```python
from build123d import *

# Parameters (mm, degrees)
BASE_BLOCK_DEPTH      = 20
BASE_RECESS_CUT_DEPTH = 75
HUB_CIRCLE_SKETCH_R   = 20
BEARING_HUB_DEPTH     = 44
SUPPORT_WEB_DEPTH     = 24
SIDE_WINDOW_CUT_DEPTH = 24
BEARING_BORE_SKETCH_R = 8
BEARING_BORE_DEPTH    = 57
SIDE_RIB_DEPTH        = 20


with BuildPart() as part:
    # Base Profile Sketch → Base Block (new body)
    with BuildSketch(Plane(origin=(0, 0, 0), x_dir=(1, 0, 0), z_dir=(0, 1, 0))):
        Polygon((30, 0), (30, 45), (-30, 45), (-30, -45), (30, -45), align=None)
    extrude(amount=BASE_BLOCK_DEPTH)

    # Base Recess Sketch → Base Recess Cut (cut)
    with BuildSketch(Plane(origin=(30, 0, 0), x_dir=(0, 0, -1), z_dir=(1, 0, 0))):
        Polygon((38, 20), (45, 0), (45, 20), align=None)
        Polygon((-38, 20), (-45, 0), (-45, 20), align=None)
    extrude(amount=-BASE_RECESS_CUT_DEPTH, mode=Mode.SUBTRACT)



with BuildPart() as body_2:
    # Hub Circle Sketch → Bearing Hub (new body)
    with BuildSketch(Plane(origin=(12, 0, 0), x_dir=(0, 0, -1), z_dir=(1, 0, 0))):
        with Locations((0, 50)):
            Circle(HUB_CIRCLE_SKETCH_R)
    extrude(amount=-BEARING_HUB_DEPTH)


with BuildPart() as part_1:
    add(part.part)

    add(body_2.part)  # Support Web merges body 2
    # Support Web Sketch → Support Web (add)
    with BuildSketch(Plane(origin=(2, 0, 0), x_dir=(0, 0, -1), z_dir=(1, 0, 0))):
        with BuildLine():
            Line((25, 20), (-25, 20))
            Line((-25, 20), (-38, 20))
            Line((-38, 20), (-25, 58))
            Line((-25, 58), (-18.33030278, 58))
            ThreePointArc((-18.33030278, 58), (0, 30), (18.33030278, 58))
            Line((18.33030278, 58), (25, 58))
            Line((25, 58), (38, 20))
            Line((38, 20), (25, 20))
        make_face()
    extrude(amount=-SUPPORT_WEB_DEPTH)

    # Side Window Sketch → Side Window Cut (cut)
    with BuildSketch(Plane(origin=(2, 0, 0), x_dir=(0, 0, -1), z_dir=(1, 0, 0))):
        with BuildLine():
            Line((-8, 68.33030278), (-8, 58))
            Line((-8, 58), (-18.33030278, 58))
            ThreePointArc((-18.33030278, 58), (-14.142135624, 64.142135624), (-8, 68.33030278))
        make_face()
    side_window_cut = extrude(amount=-SIDE_WINDOW_CUT_DEPTH, mode=Mode.SUBTRACT)

    # Side Window Mirror: Side Window Cut across plane
    add(side_window_cut.mirror(Plane.XY), mode=Mode.SUBTRACT)

    # Bearing Bore Sketch → Bearing Bore (cut)
    with BuildSketch(Plane(origin=(12, 0, 0), x_dir=(0, 0, -1), z_dir=(1, 0, 0))):
        with Locations((0, 50)):
            Circle(BEARING_BORE_SKETCH_R)
    extrude(amount=-BEARING_BORE_DEPTH, mode=Mode.SUBTRACT)

    # Side Rib Sketch → Side Rib (add)
    with BuildSketch(Plane.XY.offset(45)):
        Polygon((-10, 7), (-2, 7), (-2, 45), (-18, 45), (-18, 7), align=None)
    side_rib = extrude(amount=-SIDE_RIB_DEPTH)

    # Side Rib Mirror: Side Rib across plane
    add(side_rib.mirror(Plane.XY))


solid = part_1.part
```
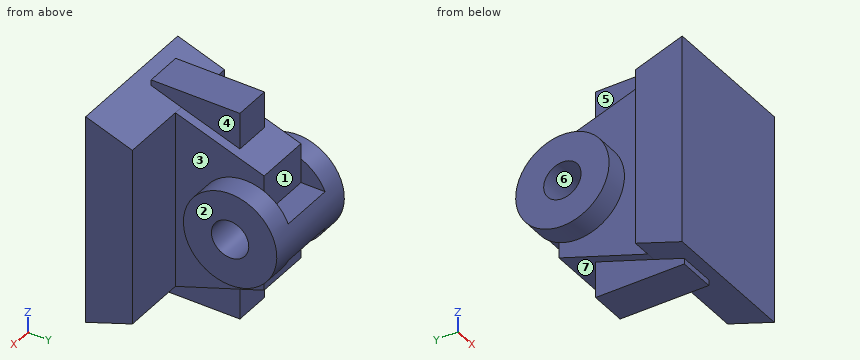
Design review of the part built by this model. Coordinates are the model's own, in mm. Face numbers are marked on the shaded views. A direction names the side the tool comes from. Give positions to 0.01 mm unless a question says otherwise; leave off trailing zeros. Write each loop counter-clockwise with the first axis right and the second up, starting at its lowest first coordinate (ties: lowest second). Pieces come first, ordered by that corner, then holes.
(1) Add section A-A (y = 16). Give the boundary of the cut face in (x, z).
Checked values:
outline: (-30, -39.4) - (-18, -39.4) - (-18, -45) - (-2, -45) - (-2, -39.4) - (30, -39.4) - (30, 39.4) - (-2, 39.4) - (-2, 45) - (-18, 45) - (-18, 39.4) - (-30, 39.4) - close
(2) Mouldability with a two-part tool opening along Y and no side actions: class the marked faces 5, 6 and 7 as +Y half, -Y half, draft (parallel to the pull), parting line (faces both ways), or undercut.
Checked values:
face 5: draft
face 6: undercut
face 7: +Y half
(3) Clearance check with flat-ended pins moving along their axes: pin 1 Ø10 at (x, z) = (9.5, 10) entering from +Y; pin 2 Ø6 at (y, z) = (38, -31.5) entering from +X; pin 3 Ø17 at (x, z) = (-9, -38.5) entering from +Y. State where each tip first meets the part, or that it passes through.
Checked values:
pin 1: stops at y = 69.36
pin 2: stops at x = 2
pin 3: stops at y = 45
(4) Add section C-C (y = 50). Give the boundary of the cut face in (x, z).
Checked values:
outline: (-32, -20) - (-22, -20) - (-22, -27.74) - (2, -27.74) - (2, -20) - (12, -20) - (12, -8) - (-32, -8) - close; (-32, 8) - (12, 8) - (12, 20) - (2, 20) - (2, 27.74) - (-22, 27.74) - (-22, 20) - (-32, 20) - close
(5) Add section B-B (z = 0). Give the boundary of the cut face in (x, y), and give its area (3 significant figures).
Checked values:
outline: (-32, 30) - (-22, 30) - (-22, 20) - (-30, 20) - (-30, 0) - (30, 0) - (30, 20) - (2, 20) - (2, 30) - (12, 30) - (12, 42) - (-32, 42) - close; (-32, 58) - (12, 58) - (12, 70) - (-32, 70) - close
area: 2,500 mm2
(6) Tool access review of the marked faces 1, 2, 3 and 4: name each direction out of +Z, -Z, +X, -X, +Y, -Y from which nothing blocks a thin tool from reaching the whole face with its end or side.
Checked values:
face 1: +Z, +Y
face 2: +Z, -Z, +X, +Y
face 3: +X
face 4: +Z, +X, +Y
(7) Add section D-D (x = 18). Give the boundary of the cut face in (y, z).
Checked values:
outline: (0, -45) - (20, -38) - (20, 38) - (0, 45) - close
(8) Wall thickness on line 1 along Y through (x, z) = (-11, 0); line 2 along Y through (x, z) = (-29, -5) (3 decimals); line 3 along Z through (x, y) = (-9, 67): over which ranges is each line inside the solid? List them lowest first.
Checked values:
line 1: y = 0 to 42, 58 to 70
line 2: y = 0 to 20, 30.635 to 43.755, 56.245 to 69.365
line 3: z = -8 to 8
